Part model, mm, in its own coordinate system. A direction names the side the tool comes from. Coordinates: 2 decimals unless noted, no trailing zeros. Loops run counter-clockwise (first coordinate to the right, second up) from the corner with the lowest first, then second, coordinate; pieces in that order, holes last. Notation, with made-up numbers: (-17, -4) - (20, -4) arc R20 cw to (20, 8) - close; hole circle Ø2 at (-16, 48). An arc over 180 degrees is marked (long way). Use a Markdown table: item, result. Add a question column.
1. Drop flat-ended pins along their axis: pin 1 (10 mm diameter, centred on x = 15.5, y = 13.5, fed in from +Z); pin 2 (2 mm diameter, centred on x = -4, z = -9.5, fed in from +Y); pin 3 (2 mm diameter, centred on x = 4.5, z = -3.5, fed in from -Y). Give the stop position or say it passes through.
2. 3-axis set-ups, long thin cutter, end or side, ignore diameter. For faces 1 (the cylindrical face through (8.06, -12.65, -2.96)), 2 (the conical face through (5.453, -1.717, -9.125)): which of +Z, -Z, +X, -X, +Y, -Y reach the whole face in a straight line?
3. Band-saw the part on A-A, the plane y = 0. Give the cut face in (x, z).
4. Band-saw the part on D-D, the plane x = -10. Give the cut face in (y, z), plus the area to 3 significant figures.
5. Band-saw the part on C-C, the plane z = -3.25. Give the cut face in (x, y).
6. Wall check: probe 1 along Z at (x, y) = (16, -9); probe 2 along Y at (x, z) = (0, -6.5); probe 3 along Y at (x, z) = (0, -4.5). Give the ranges that are in metal, low to high. Write a range as [from, to].
from build123d import *


with BuildPart() as part:
    # Sketch1 → Revolve1 (revolve)
    with BuildSketch(Plane(origin=(0, 0, 0), x_dir=(0, 0, -1), z_dir=(1, 0, 0)), mode=Mode.PRIVATE) as revolve1_sk:
        Polygon((0, 15), (0, 5.5), (9, 5.5), (11, 8.964101615), (11, 22), (6, 22), (6, 15), align=None)
    revolve(revolve1_sk.sketch.rotate(Axis((0, 0, 17.908444602), (0, 0, -1)), 90), axis=Axis((0, 0, 17.908444602), (0, 0, -1)))


solid = part.part
Geometry check:
| question | item | result |
|---|---|---|
| 1 | pin 1 | stops at z = -6 |
| 1 | pin 2 | stops at y = 21.79 |
| 1 | pin 3 | stops at y = -14.59 |
| 2 | face 1 | +Z |
| 2 | face 2 | -Z |
| 3 | outline | (-22, -11) - (-8.96, -11) - (-5.5, -9) - (-5.5, 0) - (-15, 0) - (-15, -6) - (-22, -6) - close; (5.5, -9) - (8.96, -11) - (22, -11) - (22, -6) - (15, -6) - (15, 0) - (5.5, 0) - close |
| 4 | outline | (-19.6, -11) - (19.6, -11) - (19.6, -6) - (11.18, -6) - (11.18, 0) - (-11.18, 0) - (-11.18, -6) - (-19.6, -6) - close |
| 4 | area | 330 mm^2 |
| 5 | outline | circle Ø30 at (0, 0); hole circle Ø11 at (0, 0) |
| 6 | probe 1 | z = [-11, -6] |
| 6 | probe 2 | y = [-22, -5.5], [5.5, 22] |
| 6 | probe 3 | y = [-15, -5.5], [5.5, 15] |
